The model under review builds one solid part; all positions refer to its coordinate system, in mm. Coordinates: 2 decimals unless noted, no trailing zeros. Loops run counter-clockwise (first coordinate to the right, second up) from the corner with the lowest first, then second, coordinate; pieces in that order, holes last. Notation, with made-up numbers: (-5, 45) - (49, 45) arc R12 ccw to (49, 65) - close; hole circle Ø4 at (75.5, 87.25). An arc over 180 degrees is marked (long way). One line per item, written item: value. Start each with the question number.
1. Insertion check: P1, Ø1.5, axis at x = -8.5, y = -5, coming from the -Z side. The pin has a flat end and moves straight along its axis. Give the tip position at first contact, or say it passes through.
2. We need section C-C, the plane z = 1.6. Give the boundary of the cut face in (x, y).
3. We need section A-A, the plane x = -15. Give the boundary of the cut face in (y, z), then the cut area to 3 significant figures.
4. We need section B-B, the plane y = 0. Give the boundary of the cut face in (x, z), then the cut area to 3 significant figures.
5. To check wall thickness, follow line 1 (Y direction, x = 15, z = 1.25); line 2 (X direction, y = -1.5, z = 1.5); line 3 (X direction, y = -1, z = 0.3). State the ranges of each line that lie inside material, in increasing order.
6. Mouldability with a two-part tool opening along X and no side actions: class faces 1 (the face through (0, 0, 0)), 2 (the face through (-13.331, 0.526, 1.479)), 3 (the face through (19.5, 0, 1)), 4 (the face through (16.669, 0.526, 1.479)) as +X half, -X half, draft (parallel to the pull), parting line (faces both ways), or undercut.
7. We need section D-D, the plane x = 14.5. Give the boundary of the cut face in (y, z), then the cut area to 3 significant figures.
from build123d import *

# Parameters (mm, degrees)
SKETCH1_W           = 39
SKETCH1_H           = 20
SKETCH1_R           = 1.75
BOSS_EXTRUDE1_DEPTH = 3
CHAMFER1_SIZE       = 1


with BuildPart() as part:
    # Sketch1 → Boss-Extrude1 (new body)
    with BuildSketch(Plane.XY):
        Rectangle(SKETCH1_W, SKETCH1_H)
        with Locations((-15, 0)):
            Circle(SKETCH1_R, mode=Mode.SUBTRACT)
        with Locations((15, 0)):
            Circle(SKETCH1_R, mode=Mode.SUBTRACT)
    extrude(amount=BOSS_EXTRUDE1_DEPTH)

    # Chamfer1
    chamfer1_edges = [part.edges().sort_by_distance(p)[0] for p in [
        (19.5, -10, 1.5),
        (-19.5, -10, 1.5),
        (-19.5, 10, 1.5),
        (19.5, 10, 1.5),
    ]]
    chamfer(chamfer1_edges, length=CHAMFER1_SIZE)


solid = part.part
Findings below:
1. P1: z = 0
2. outline: (-19.5, -9) - (-18.5, -10) - (18.5, -10) - (19.5, -9) - (19.5, 9) - (18.5, 10) - (-18.5, 10) - (-19.5, 9) - close; hole circle Ø3.5 at (-15, 0); hole circle Ø3.5 at (15, 0)
3. outline: (-10, 0) - (-1.75, 0) - (-1.75, 3) - (-10, 3) - close; (1.75, 0) - (10, 0) - (10, 3) - (1.75, 3) - close
3. area: 49.5 mm2
4. outline: (-19.5, 0) - (-16.75, 0) - (-16.75, 3) - (-19.5, 3) - close; (-13.25, 0) - (13.25, 0) - (13.25, 3) - (-13.25, 3) - close; (16.75, 0) - (19.5, 0) - (19.5, 3) - (16.75, 3) - close
4. area: 96.0 mm2
5. line 1: -10 to -1.75, 1.75 to 10
5. line 2: -19.5 to -15.9, -14.1 to 14.1, 15.9 to 19.5
5. line 3: -19.5 to -16.44, -13.56 to 13.56, 16.44 to 19.5
6. face 1: draft
6. face 2: undercut
6. face 3: +X half
6. face 4: undercut
7. outline: (-10, 0) - (-1.68, 0) - (-1.68, 3) - (-10, 3) - close; (1.68, 0) - (10, 0) - (10, 3) - (1.68, 3) - close
7. area: 49.9 mm2
